Input: part model. Units: mm. Frame: model coordinates. A direction names the side the tool comes from. Give positions to 0.01 mm unless a question says otherwise; leave off trailing zeros. Loops run counter-clockwise (first coordinate to the right, second up) from the corner with the lowest first, then second, coordinate; pieces in that order, holes last. Notation, with made-up numbers: (13.5, 84.5) - (54.5, 84.5) arc R35 ccw to (54.5, 119.5) - close; hole circle Ø6 at (14.5, -9). An arc over 180 degrees is marked (long way). Answer as a JSON object with one key per item and string values. Group by question number.
(1) Access query for faces 4 (the cylindrical face through (581.274, 209.849, -1049.763)), 5 (the conical face through (510.55, 186.67, -1067.02)), 6 (the flat face through (463, 235, -1054.693)). Directions: +Z, -Z, +X, -X, +Y, -Y. A direction counts if a zero-diameter tool reaches every point of the face in a straight line with its end or side. Return the directions, or none.
(2) Section query A-A (x = 576.5). Return loops of the section in (y, z).
(3) Section query B-B (z = -1077.5). Return loops of the section in (x, y).
(4) Mould query, pull axis Z, two halves, no side actions, for faces 1 (the cylindrical face through (475.204, 199.452, -1057.228)), 2 (the cylindrical face through (508.22, 176.17, -1079.97)), 3 (the flat face through (489.8, 195, -1099.693)). Classes: +Z half, -Z half, draft (parallel to the pull), parting line (faces both ways), or undercut.
(5) Section query C-C (z = -1070). Return loops of the section in (x, y).
(6) Pin query (flat end, axial travel): P1, Ø10, axis at x = 561, z = -1055.5, coming from the -Y side; P2, Ø12, axis at x = 526.5, z = -1051, coming from the +Y side; P3, Ø10, axis at x = 518, z = -1077, coming from the +Y side. Return the tip coordinate at first contact, or that it passes through.
(7) Material intervals for L1, parallel to X at y = 214.5, z = -1073; L2, parallel to Y at x = 546.5, z = -1092; L3, parallel to Y at x = 554, z = -1082.5, sorted ascending.
```python
from build123d import *


with BuildPart() as part:
    # Sketch1 → Revolve1 (revolve)
    with BuildSketch(Plane(origin=(0, 234.743963655, 0), x_dir=(1, 0, 0), z_dir=(0, 1, 0))):
        Polygon((586.230642584, 1054.692956355), (579.230642584, 1054.692956355), (579.230642584, 1059.692956355), (581.230642584, 1059.692956355), (581.230642584, 1099.692956355), (571.730642584, 1099.692956355), (570.730642584, 1079.692956355), (570.230642584, 1054.692956355), (572.480642584, 1044.692956355), (586.230642584, 1044.692956355), align=None)
    revolve(axis=Axis((521.230642584, 234.743963655, -1099.692956355), (0, 0, 1)))


solid = part.part
```
Recorded:
{
 "1": {"face 4": "+Z, -Z", "face 5": "-Z", "face 6": "none"},
 "2": {"outline": "(200.53, -1054.69) - (217.16, -1054.69) - (217.16, -1059.69) - (211.39, -1059.69) - (211.39, -1099.69) - (258.1, -1099.69) - (258.1, -1059.69) - (252.33, -1059.69) - (252.33, -1054.69) - (268.95, -1054.69) - (268.95, -1044.69) - (200.53, -1044.69) - close"},
 "3": {"outline": "circle Ø120 at (521.23, 234.74); hole circle Ø98.91 at (521.23, 234.74)"},
 "4": {"face 1": "undercut", "face 2": "draft", "face 3": "-Z half"},
 "5": {"outline": "circle Ø120 at (521.23, 234.74); hole circle Ø98.61 at (521.23, 234.74)"},
 "6": {"P1": "stops at y = 179.87", "P2": "stops at y = 299.74", "P3": "stops at y = 294.74"},
 "7": {"L1": "x = 464.75 to 476.21, 566.26 to 577.71", "L2": "y = 180.32 to 191.47, 278.02 to 289.16", "L3": "y = 184.48 to 197.46, 272.03 to 285"}
}
